from build123d import *

# Parameters (mm, degrees)
SKETCH1_W                  = 28
SKETCH1_H                  = 24
BOSS_EXTRUDE1_DEPTH        = 0.75
FILLET1_R                  = 4
F_3_5_3_5_DIAMETER_HOLE1_D = 3.5
F_1_0_1_DIAMETER_HOLE1_D   = 1
LPATTERN1_COUNT            = 6
LPATTERN1_PITCH            = 3
LPATTERN1_COUNT_DIR2       = 7
LPATTERN1_PITCH_DIR2       = 3


with BuildPart() as part:
    # Sketch1 → Boss-Extrude1 (new, symmetric)
    with BuildSketch(Plane.XY):
        Rectangle(SKETCH1_W, SKETCH1_H)
    extrude(amount=BOSS_EXTRUDE1_DEPTH, both=True)

    # Fillet1
    fillet1_edges = [part.edges().sort_by_distance(p)[0] for p in [
        (14, -12, 0),
        (-14, -12, 0),
        (-14, 12, 0),
        (14, 12, 0),
    ]]
    fillet(fillet1_edges, radius=FILLET1_R)

    # Ø3.5 (3.5) Diameter Hole1 (through all)
    with Locations(Plane.XY.offset(0.75)):
        with Locations((-10.5, 6), (-10.5, -6)):
            Hole(F_3_5_3_5_DIAMETER_HOLE1_D / 2)

    # Ø1.0 (1) Diameter Hole1 (through all)
    with Locations(Plane.XY.offset(0.75)):
        with Locations((10, -9)):
            f_1_0_1_diameter_hole1 = Hole(F_1_0_1_DIAMETER_HOLE1_D / 2)

    # LPattern1: 1.0 _1_ Diameter Hole1 6 × 7
    with Locations(*[(-i * LPATTERN1_PITCH, j * LPATTERN1_PITCH_DIR2, 0) for i in range(LPATTERN1_COUNT) for j in range(LPATTERN1_COUNT_DIR2) if (i, j) != (0, 0)]):
        add(f_1_0_1_diameter_hole1, mode=Mode.SUBTRACT)


solid = part.part
Work out the finished part from the listing and answer in its coordinate system (mm). Give positions to 0.01 mm unless a question says otherwise; leave off trailing zeros. Loops run counter-clockwise (first coordinate to the right, second up) from the corner with the lowest first, then second, coordinate; pieces in that order, holes last. Notation, with made-up numbers: (52, 36.25) -> (104, 36.25) arc R28 ccw to (104, 75.25) -> close; hole circle Ø11 at (37.5, 51). An arc over 180 degrees is marked (long way). Use a Markdown table: item, result. Add a question column.
1. A flat-ended cylindrical pin translates along its axis: pin 1 Ø4.5 at (x, y) = (-10.5, -6) entering from -Z. Find the tip coordinate at first contact, or state that the pin passes through.
2. Section A-A on y = -6 is taken. State how many separate pieces and enclosed holes the cut face has, and give its area (4 significant figures).
3. Section C-C on x = -10.5 is taken. Determine the outline of the cut face in (y, z), and give its area (3 significant figures).
4. Determine the mould class of faces 1 (the flat face through (0, 12, 0)), 2 (the flat face through (-14, 0, 0)), 3 (the cylindrical face through (10.4, 5.7, 0)) for opening direction X: released by +X, released by -X, zero draft, split by the parting line, or undercut.
5. Find the intervals of material crossed by probe 1 along Y at (x, z) = (-9.75, -0.6); probe 2 along X at (y, z) = (-7.25, -0.6); probe 3 along Y at (x, z) = (-10.5, 0.05), in increasing order.
Results below:
| question | item | result |
|---|---|---|
| 1 | pin 1 | stops at z = -0.75 |
| 2 | separate pieces | 8 |
| 2 | enclosed holes | 0 |
| 2 | area | 27.75 mm^2 |
| 3 | outline | (-11.97, -0.75) -> (-7.75, -0.75) -> (-7.75, 0.75) -> (-11.97, 0.75) -> close; (-4.25, -0.75) -> (4.25, -0.75) -> (4.25, 0.75) -> (-4.25, 0.75) -> close; (7.75, -0.75) -> (11.97, -0.75) -> (11.97, 0.75) -> (7.75, 0.75) -> close |
| 3 | area | 25.4 mm^2 |
| 4 | face 1 | zero draft |
| 4 | face 2 | released by -X |
| 4 | face 3 | undercut |
| 5 | probe 1 | y = -12 to -7.58, -4.42 to 4.42, 7.58 to 12 |
| 5 | probe 2 | x = -14 to -11.72, -9.28 to 14 |
| 5 | probe 3 | y = -11.97 to -7.75, -4.25 to 4.25, 7.75 to 11.97 |
